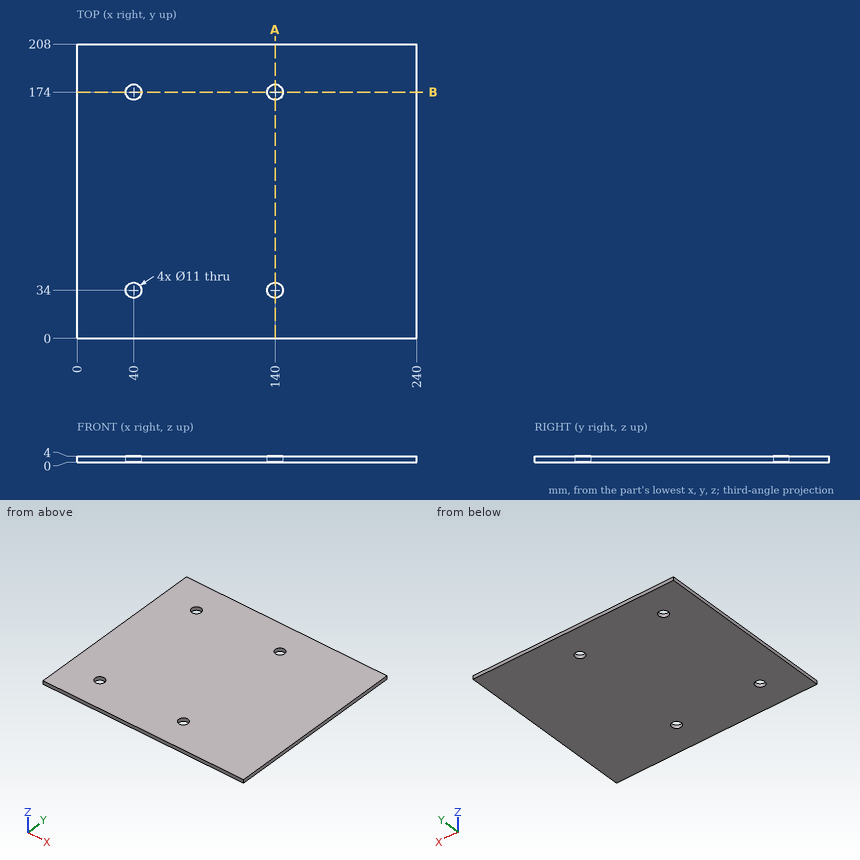
Geometry: see drawing. Coordinates: mm, zero at the bounding-box minimum. Coordinates: 2 decimals unless noted, no trailing zeros. Loops run counter-clockwise (first coordinate to the right, second up) from the corner with the lowest first, then second, coordinate; pieces in that order, holes last. Notation, with made-up numbers: (-27, -37) -> (18, -37) arc R19 cw to (18, -19) -> close; hole circle Ø8 at (-17.75, -13). An arc over 180 degrees is marked (long way). Use a Markdown table: item, result.
1) Cut plane B-B (y = 174). Return the cut outline in (x, z), then the cut area to 3 significant figures.
Results found:
| item | result |
|---|---|
| outline | (0, 0) -> (34.5, 0) -> (34.5, 4) -> (0, 4) -> close; (45.5, 0) -> (134.5, 0) -> (134.5, 4) -> (45.5, 4) -> close; (145.5, 0) -> (240, 0) -> (240, 4) -> (145.5, 4) -> close |
| area | 872 mm2 |
2) Contact query for a flat-ended pin moving along its axis: pin 1 (17.5 mm diameter, centred on x = 140, y = 34, fed in from -Z). Output: stop coordinate, or through.
Results found:
| item | result |
|---|---|
| pin 1 | stops at z = 0 |
3) Cut plane A-A (x = 140). Return the cut outline in (y, z).
Results found:
| item | result |
|---|---|
| outline | (0, 0) -> (28.5, 0) -> (28.5, 4) -> (0, 4) -> close; (39.5, 0) -> (168.5, 0) -> (168.5, 4) -> (39.5, 4) -> close; (179.5, 0) -> (208, 0) -> (208, 4) -> (179.5, 4) -> close |
4) Material intervals for line 1 along Y through (x, z) = (40, 2.2); line 2 along X through (y, z) = (174, 1), sorted ascending. Write a range as from..to.
Results found:
| item | result |
|---|---|
| line 1 | y = 0..28.5, 39.5..168.5, 179.5..208 |
| line 2 | x = 0..34.5, 45.5..134.5, 145.5..240 |
